The model under review builds one solid part; all positions refer to its coordinate system, in mm. A direction names the side the tool comes from. Coordinates: 2 decimals unless noted, no trailing zeros. Loops run counter-clockwise (first coordinate to the right, second up) from the corner with the lowest first, then second, coordinate; pieces in that order, holes last. Notation, with made-up numbers: M 72,76.25 L 116,76.25 A19 cw 116,89.25 Z; hole C -20,83.25 d4. An arc over 180 degrees is marked long. One line per item, written item: value.
```python
from build123d import *

# Parameters (mm, degrees)
SKETCH1_R                   = 9
BOSS_EXTRUDE1_DEPTH         = 69.5
SKETCH2_R                   = 7
CUT_EXTRUDE1_DEPTH          = 32
CUT_EXTRUDE3_START          = -35
SKETCH3_R                   = 9
SKETCH3_R_2                 = 8.5
CUT_EXTRUDE3_DEPTH          = 1
CUT_EXTRUDE4_START          = -7
SKETCH4_R                   = 9
SKETCH4_R_2                 = 8.5
CUT_EXTRUDE4_DEPTH          = 1
CUT_EXTRUDE5_START          = -7
SKETCH5_R                   = 9
SKETCH5_R_2                 = 8.5
CUT_EXTRUDE5_DEPTH          = 1
M5_TAPPED_HOLE1_D           = 4.2
M5_TAPPED_HOLE1_DEPTH       = 8.7381927
M5_TAPPED_HOLE1_CSINK_D     = 5.05
M5_TAPPED_HOLE1_CSINK_ANGLE = 90
M5_TAPPED_HOLE1_TIP         = 1.2618073


with BuildPart() as part:
    # Sketch1 → Boss-Extrude1 (new body)
    with BuildSketch(Plane.XY):
        Circle(SKETCH1_R)
    extrude(amount=BOSS_EXTRUDE1_DEPTH)

    # Sketch2 → Cut-Extrude1 (cut)
    with BuildSketch(Plane(origin=(0, 0, 0), x_dir=(-1, 0, 0), z_dir=(0, 0, -1))):
        Circle(SKETCH2_R)
    extrude(amount=-CUT_EXTRUDE1_DEPTH, mode=Mode.SUBTRACT)

    # Sketch3 → Cut-Extrude3 (cut)
    with BuildSketch(Plane(origin=(0, 0, 0), x_dir=(-1, 0, 0), z_dir=(0, 0, -1)).offset(CUT_EXTRUDE3_START)):
        Circle(SKETCH3_R)
        Circle(SKETCH3_R_2, mode=Mode.SUBTRACT)
    extrude(amount=-CUT_EXTRUDE3_DEPTH, mode=Mode.SUBTRACT)

    # Sketch4 → Cut-Extrude4 (cut)
    with BuildSketch(Plane(origin=(0, 0, 36), x_dir=(-1, 0, 0), z_dir=(0, 0, -1)).offset(CUT_EXTRUDE4_START)):
        Circle(SKETCH4_R)
        Circle(SKETCH4_R_2, mode=Mode.SUBTRACT)
    extrude(amount=-CUT_EXTRUDE4_DEPTH, mode=Mode.SUBTRACT)

    # Sketch5 → Cut-Extrude5 (cut)
    with BuildSketch(Plane(origin=(0, 0, 44), x_dir=(-1, 0, 0), z_dir=(0, 0, -1)).offset(CUT_EXTRUDE5_START)):
        Circle(SKETCH5_R)
        Circle(SKETCH5_R_2, mode=Mode.SUBTRACT)
    extrude(amount=-CUT_EXTRUDE5_DEPTH, mode=Mode.SUBTRACT)

    # Sketch6 → Revolve1 (revolve)
    with BuildSketch(Plane(origin=(0, 0, 0), x_dir=(1, 0, 0), z_dir=(0, 1, 0))):
        with BuildLine():
            Line((0, -69.5), (0, -71.99166898))
            ThreePointArc((0, -71.99166898), (-4.669272275, -71.357252173), (-9, -69.5))
            Line((-9, -69.5), (0, -69.5))
        make_face()
    revolve(axis=Axis((0, 0, 0), (0, 0, 1)))

    # M5 Tapped Hole1
    with Locations(Plane(origin=(0, 0, 32), x_dir=(-1, 0, 0), z_dir=(0, 0, -1))):
        with Locations((0, 0)):
            CounterSinkHole(M5_TAPPED_HOLE1_D / 2, M5_TAPPED_HOLE1_CSINK_D / 2, depth=M5_TAPPED_HOLE1_DEPTH, counter_sink_angle=M5_TAPPED_HOLE1_CSINK_ANGLE)
            with Locations((0, 0, -(M5_TAPPED_HOLE1_DEPTH + M5_TAPPED_HOLE1_TIP / 2))):  # 118° drill point
                Cone(0, M5_TAPPED_HOLE1_D / 2, M5_TAPPED_HOLE1_TIP, mode=Mode.SUBTRACT)


solid = part.part
```
(1) Tool access review of faces 4 (the face through (-4.57, 7.167, 35.493)), 5 (the face through (-1.172, 8.923, 17.255)), 6 (the face through (-6.466, -2.681, 15.776)): name each direction out of +Z, -Z, +X, -X, +Y, -Y from which nothing blocks a thin tool from reaching the whole face with its end or side.
Checks:
face 4: none
face 5: +Z, -Z
face 6: -Z
(2) Add section A-A on z = 12.5. State the section outline as (x, y) points.
Checks:
outline: C 0,0 d18; hole C 0,0 d14
(3) To check wall thickness, follow L1, parallel to Y at x = 0, z = 37.25; L2, parallel to Y at x = 0, z = 18. State the ranges of each line that lie inside material, in increasing order. Write a range as [from, to].
Checks:
L1: [-9, -2.1], [2.1, 9]
L2: [-9, -7], [7, 9]
(4) Add section C-C on z = 46. State the section outline as (x, y) points.
Checks:
outline: C 0,0 d18
(5) Draft analysis for pull direction Y (two halves, no side actions). For faces 1 (the face through (-1.172, 8.923, 60.628)), 2 (the face through (-3.3, -8, 44)), 3 (the face through (2.003, 0.631, 36.64)), state which applies: pulls with the +Y half, pulls with the -Y half, needs draft (parallel to the pull), parting line crosses it, or undercut.
Checks:
face 1: parting line crosses it
face 2: needs draft
face 3: undercut
(6) Insertion check: pin 1 Ø1 at (y, z) = (-3, 26) entering from -X; pin 2 Ø1.5 at (x, y) = (-2, 5) entering from -Z; pin 3 Ø1 at (x, y) = (-0.5, 1.5) entering from +Z. Each pin has a flat end and moves straight along its axis. Give the tip position at first contact, or say it passes through.
Checks:
pin 1: x = -8.65
pin 2: z = 32
pin 3: z = 71.96
